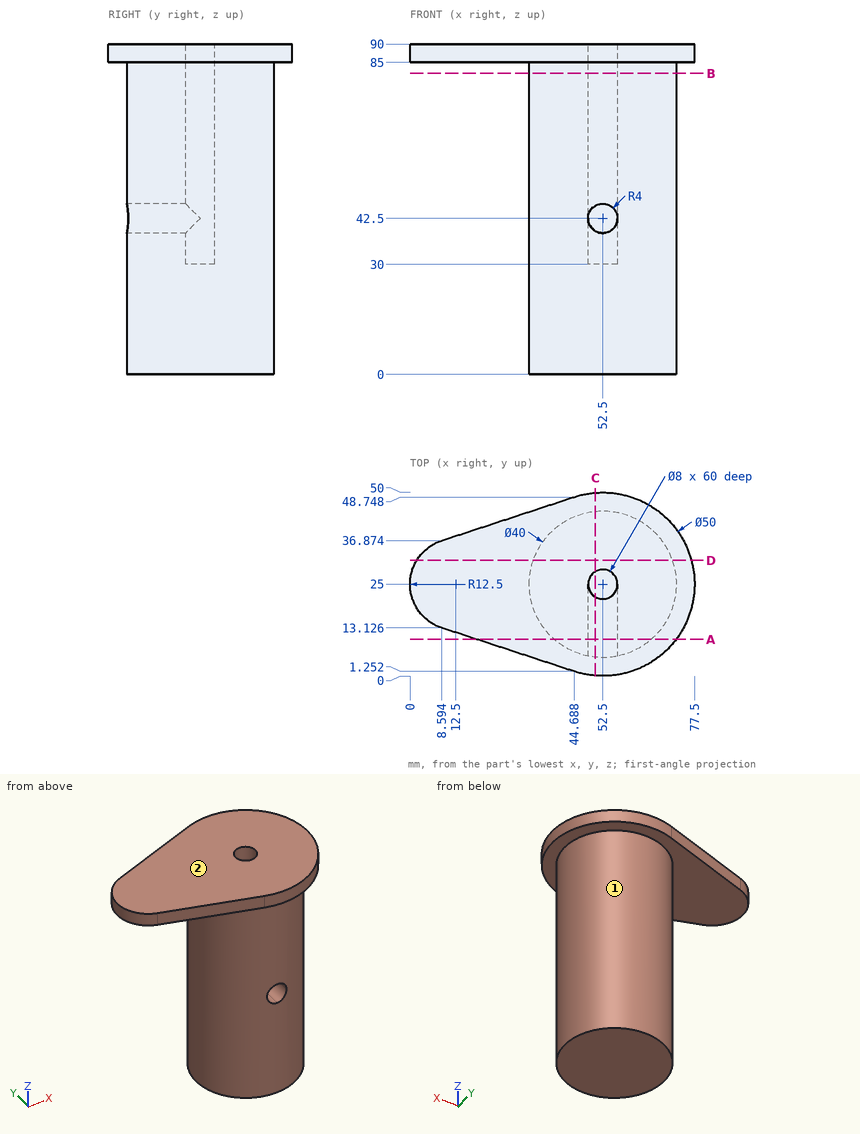
Part print with two shaded views. Sizes in mm from the minimum x, y, z corner. A direction names the side the tool comes from. Give positions to 0.01 mm unless a question says otherwise; leave off trailing zeros. Loops run counter-clockwise (first coordinate to the right, second up) from the corner with the lowest first, then second, coordinate; pieces in that order, holes last. Notation, with made-up numbers: (-35.5, 39.5) -> (-23.5, 39.5) arc R12 ccw to (-23.5, 53.5) -> close; hole circle Ø11 at (10.5, 83). An arc over 180 degrees is marked (long way). One line per question, with ' | ' between items.
Q1. Drop flat-ended pins along their axis: pin 1 (4 mm diameter, centred on y = 39.5, z = 52.5, fed in from -X); pin 2 (2 mm diameter, centred on y = 32.5, z = 29.5, fed in from -X) (1 decimal); pin 3 (3 mm diameter, centred on y = 41.5, z = 68.5, fed in from +X). Give the stop position or say it passes through.
Filled sheet:
pin 1: stops at x = 36.89 | pin 2: stops at x = 33.6 | pin 3: stops at x = 65.73
Q2. Drill centre lines: line 1 along Y through (x, z) = (52.5, 49.5); line 2 along Z through (x, y) = (52.5, 24); line 3 along Z through (x, y) = (27.5, 20). Where is each one in solid material? Low to high. Write a range as [from, to].
Filled sheet:
line 1: y = [5, 21], [29, 45] | line 2: z = [0, 30] | line 3: z = [85, 90]
Q3. Tool access for the marked faces 1 and 2: list every direction of +Z, -Z, +X, -X, +Y, -Y with a clear straight run to the whole face (end or side of a thin tool).
Filled sheet:
face 1: -Z | face 2: +Z, +X, -X, +Y, -Y
Q4. Cut at D-D, the plane y = 31.5. Write the cut outline in (x, z) (1 decimal).
Filled sheet:
outline: (1.8, 85) -> (33.6, 85) -> (33.6, 0) -> (71.4, 0) -> (71.4, 85) -> (76.6, 85) -> (76.6, 90) -> (1.8, 90) -> close
Q5. Cut at B-B, the plane z = 82. Write the cut outline in (x, y), plus the area to 3 significant figures.
Filled sheet:
outline: circle Ø40 at (52.5, 25); hole circle Ø8 at (52.5, 25) | area: 1,210 mm²
Q6. Cut at C-C, the plane x = 50.5. Write the cut outline in (y, z) (1 decimal), plus the area to 3 significant figures.
Filled sheet:
outline: (0.1, 85) -> (5.1, 85) -> (5.1, 46) -> (21.5, 46) -> (21.5, 90) -> (0.1, 90) -> close; (5.1, 0) -> (44.9, 0) -> (44.9, 85) -> (49.9, 85) -> (49.9, 90) -> (28.5, 90) -> (28.5, 30) -> (21.5, 30) -> (21.5, 39) -> (5.1, 39) -> close | area: 3,100 mm²
Q7. Cut at A-A, the plane y = 10. Write the cut outline in (x, z), plus the area to 3 significant figures.
Filled sheet:
outline: (18.1, 85) -> (39.27, 85) -> (39.27, 0) -> (65.73, 0) -> (65.73, 85) -> (72.5, 85) -> (72.5, 90) -> (18.1, 90) -> close; hole circle Ø8 at (52.5, 42.5) | area: 2,470 mm²
